Can you work these out from the drawing? Everything is in mm from the part's minimum corner. A direction names the side the tool comes from. Coordinates: 2 decimals unless noted, no trailing zeros. Order: outer loops, then holes, each group sorted by start corner. A loop starts at its lowest first (then second) coordinate and runs counter-clockwise, first axis right, second up. Notation, with made-up numbers: (67.5, -7.5) - (72.5, -7.5) arc R20 cw to (72.5, 5.5) - close; hole circle Ø11 at (86.25, 61). An arc over 180 degrees is marked (long way). One line per item, written item: value.
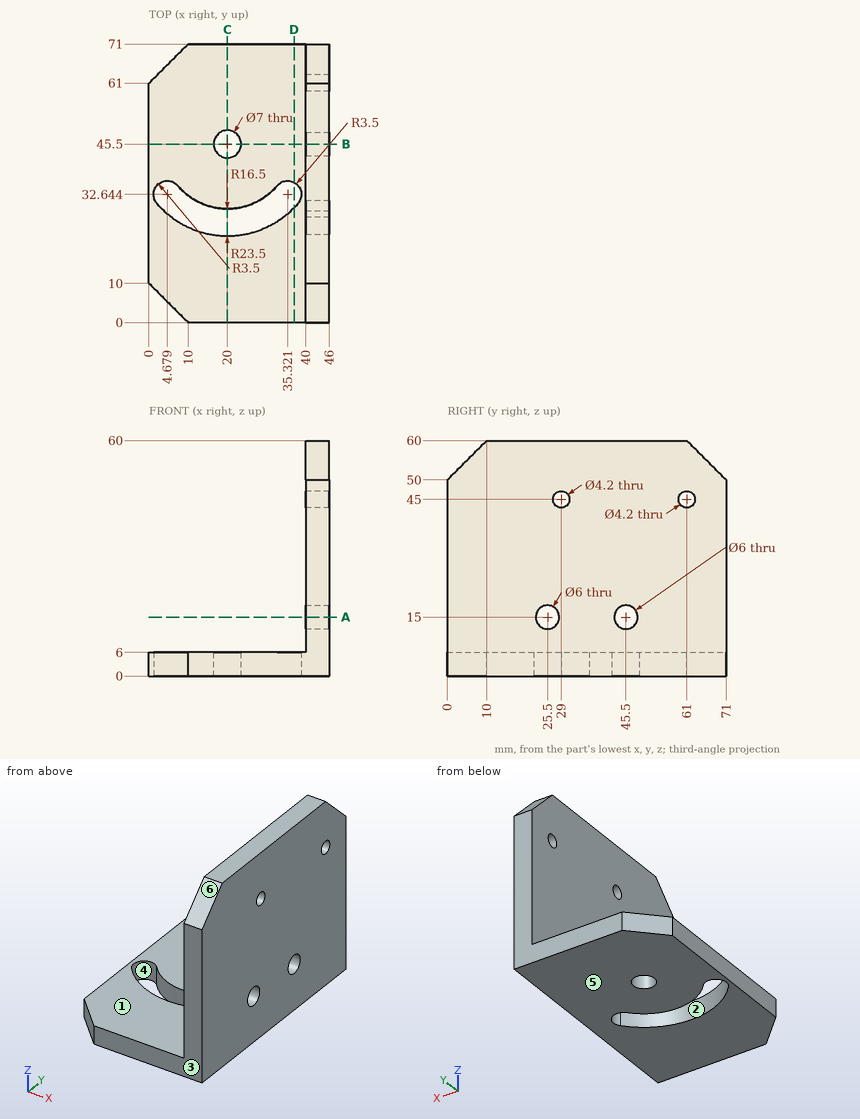
Item 1: I want a section at A-A on z = 15. Please give me the cut outline in (x, y).
Conclusion:
outline: (40, 0) - (46, 0) - (46, 22.5) - (40, 22.5) - close; (40, 28.5) - (46, 28.5) - (46, 42.5) - (40, 42.5) - close; (40, 48.5) - (46, 48.5) - (46, 71) - (40, 71) - close
Item 2: For the marked faces 1, 2 and 3, which set-ups out of +Z, -Z, +X, -X, +Y, -Y let a thin tool reach every point of the face, with its end or its side?
Conclusion:
face 1: +Z, -X, +Y, -Y
face 2: +Z, -Z
face 3: +Z, -Z, +X, -X, -Y
Item 3: Thinking about a two-plate mould opening in Y: for the marked faces 4, 5 and 6, which applies, pulls with the +Y half, pulls with the -Y half, needs draft (parallel to the pull), parting line crosses it, or undercut?
Conclusion:
face 4: undercut
face 5: needs draft
face 6: pulls with the -Y half
Item 4: If I drill on probe 1 along Y at (x, z) = (20, 4.85); probe 2 along Y at (x, z) = (44, 45); probe 3 along X at (y, z) = (58.5, 32), over which ranges is the centre line in solid material (lowest first)?
Conclusion:
probe 1: 0 to 22, 29 to 42, 49 to 71
probe 2: 0 to 26.9, 31.1 to 58.9, 63.1 to 71
probe 3: 40 to 46
Item 5: I'm going to push flat-ended pins straight in: pin 1 Ø6 at (y, z) = (19, 16) entering from -X; pin 2 Ø3.5 at (y, z) = (61, 45) entering from +X; pin 3 Ø6 at (x, y) = (18, 21.5) entering from +Z. Where does each tip first touch, or does it pass through?
Conclusion:
pin 1: x = 40
pin 2: through
pin 3: z = 6
Item 6: I want a section at B-B on y = 45.5. Please give me the cut outline in (x, z), then the cut area to 3 significant figures.
Conclusion:
outline: (0, 0) - (16.5, 0) - (16.5, 6) - (0, 6) - close; (23.5, 0) - (46, 0) - (46, 12) - (40, 12) - (40, 6) - (23.5, 6) - close; (40, 18) - (46, 18) - (46, 60) - (40, 60) - close
area: 522 mm²
Item 7: I want a section at D-D on x = 37. Please give me the cut outline in (y, z) (1 decimal).
Conclusion:
outline: (0, 0) - (29.3, 0) - (29.3, 6) - (0, 6) - close; (35.7, 0) - (71, 0) - (71, 6) - (35.7, 6) - close
Item 8: I want a section at C-C on x = 20. Please give me the cut outline in (y, z), then the cut area to 3 significant figures.
Conclusion:
outline: (0, 0) - (22, 0) - (22, 6) - (0, 6) - close; (29, 0) - (42, 0) - (42, 6) - (29, 6) - close; (49, 0) - (71, 0) - (71, 6) - (49, 6) - close
area: 342 mm²
